Model file for the job. Use its own axes, mm. A direction names the side the tool comes from. Coordinates: 2 decimals unless noted, no trailing zeros. Order: outer loops, then holes, each group sorted by start corner. A loop starts at its lowest first (then second) coordinate and runs counter-clockwise, first axis right, second up. Notation, with made-up numbers: (-31, -2.75) -> (11, -2.75) arc R21 ccw to (11, 7.25) -> close; hole circle Ø3 at (53, 51). An arc over 180 degrees is marked (long way). Use CSV: the item, a comma, the result in double quotes. Start each with the question number.
(1) Cut at C-C on z = -9. Write the cut outline in (x, y).
(2) Pull direction X, two halves, no side cores. Call faces 1 (the cylindrical face through (-0.325, -4.536, -7.958)), 2 (the flat face through (1.485, -5.79, 2.521)), 3 (the flat face through (0, -6, -11)): pulls with the +X half, pulls with the -X half, needs draft (parallel to the pull), parting line crosses it, or undercut.
(3) Probe L1, parallel to Y at x = -0.1, z = -6.5; L2, parallel to Z at x = -0.75, y = -6.95; L3, parallel to Z at x = 0.45, y = -4.3. List the from-to ranges inside material, lowest first.
(4) Cut at A-A on x = 0. Write the cut outline in (y, z), plus the area to 3 significant figures.
(5) Tool access for faces 4 (the flat face through (-0.9, -4.8, 2.5)), 5 (the cylindrical face through (-0.33, -3.52, 1.97)), 6 (the cylindrical face through (-0.37, -7.66, -2.46)): list every direction of +Z, -Z, +X, -X, +Y, -Y with a clear straight run to the whole face (end or side of a thin tool).
(6) Cut at D-D on y = -4. Write the cut outline in (x, z).
(7) Cut at B-B on y = -5.2. Write the cut outline in (x, z), plus the area to 3 significant figures.
```python
from build123d import *

# Parameters (mm, degrees)
SKETCH_1_R          = 1.7
EXTRUDE_1_DEPTH     = 5
SKETCH_2_R          = 1.5
EXTRUDE_2_DEPTH     = 6
SKETCH_3_R          = 2.5
EXTRUDE_3_DEPTH     = 4
CUT_EXTRUDE_1_DEPTH = 3


with BuildPart() as part:
    # 草图1 → 凸台-拉伸1 (new body)
    with BuildSketch(Plane.XY):
        with Locations((0, -6)):
            Circle(SKETCH_1_R)
    extrude(amount=-EXTRUDE_1_DEPTH)

    # 草图2 → 凸台-拉伸2 (add)
    with BuildSketch(Plane(origin=(0, 0, -5), x_dir=(-1, 0, 0), z_dir=(0, 0, -1))):
        with Locations(Location((0, -6, 0), (0, 0, 180))):
            Circle(SKETCH_2_R)
    extrude(amount=EXTRUDE_2_DEPTH)

    # 草图3 → 凸台-拉伸3 (add)
    with BuildSketch(Plane.XY):
        with Locations((0, -6)):
            Circle(SKETCH_3_R)
    extrude(amount=EXTRUDE_3_DEPTH)

    # 草图4 → 切除-拉伸1 (cut)
    with BuildSketch(Plane.XY.offset(4)):
        Polygon((1.355554736, -4.921820351), (-0.255953598, -4.286965337), (-1.611508335, -5.365144986), (-1.355554737, -7.078179649), (0.255953597, -7.713034663), (1.611508334, -6.634855014), align=None)
    extrude(amount=-CUT_EXTRUDE_1_DEPTH, mode=Mode.SUBTRACT)


solid = part.part
```
Outcome:
1,outline,"circle Ø3 at (0, -6)"
2,face 1,"parting line crosses it"
2,face 2,"undercut"
2,face 3,"needs draft"
3,L1,"-7.5 to -4.5"
3,L2,"-11 to 1"
3,L3,"0 to 4"
4,outline,"(-8.5, 0) -> (-7.7, 0) -> (-7.7, -5) -> (-7.5, -5) -> (-7.5, -11) -> (-4.5, -11) -> (-4.5, -5) -> (-4.3, -5) -> (-4.3, 0) -> (-3.5, 0) -> (-3.5, 4) -> (-4.39, 4) -> (-4.39, 1) -> (-7.61, 1) -> (-7.61, 4) -> (-8.5, 4) -> close"
4,area,"45.3 mm2"
5,face 4,"+Z"
5,face 5,"+Z, -Z"
5,face 6,"-Z"
6,outline,"(-1.5, 0) -> (1.5, 0) -> (1.5, 4) -> (-1.5, 4) -> close"
7,outline,"(-2.37, 0) -> (-1.5, 0) -> (-1.5, -5) -> (-1.27, -5) -> (-1.27, -11) -> (1.27, -11) -> (1.27, -5) -> (1.5, -5) -> (1.5, 0) -> (2.37, 0) -> (2.37, 4) -> (1.4, 4) -> (1.4, 1) -> (-1.4, 1) -> (-1.4, 4) -> (-2.37, 4) -> close"
7,area,"40.8 mm2"
